```python
from build123d import *

# Parameters (mm, degrees)
SKETCH_1_W             = 42
SKETCH_1_H             = 54
EXTRUDE_1_DEPTH        = 55
SKETCH_5_W             = 65.5
SKETCH_5_H             = 65.5
EXTRUDE_3_DEPTH        = 8
SKETCH_6_R             = 10
EXTRUDE_4_DEPTH        = 5
HOLE_WIZARD_M4_1_D     = 3.3
HOLE_WIZARD_M4_1_DEPTH = 11.5
HOLE_WIZARD_M4_1_TIP   = 0.991420021
CHAMFER_1_SIZE         = 2
SKETCH_9_W             = 65.5
SKETCH_9_H             = 65.5
EXTRUDE_5_DEPTH        = 3
SKETCH_10_R            = 26
SKETCH_10_R_2          = 22.5
EXTRUDE_6_DEPTH        = 8
EXTRUDE_7_DEPTH        = 8
FILLET_1_R             = 2
FILLET_2_R             = 1
FILLET_3_R             = 0.8
SKETCH_12_R            = 1.5
CUT_EXTRUDE_1_DEPTH    = 1
CHAMFER_2_SIZE         = 2


with BuildPart() as part:
    # 草图1 → 凸台-拉伸1 (new body)
    with BuildSketch(Plane.XY):
        Rectangle(SKETCH_1_W, SKETCH_1_H)
    extrude(amount=EXTRUDE_1_DEPTH)

    # 草图5 → 凸台-拉伸3 (add)
    with BuildSketch(Plane.XY.offset(55)):
        Rectangle(SKETCH_5_W, SKETCH_5_H)
    extrude(amount=EXTRUDE_3_DEPTH)

    # 草图6 → 凸台-拉伸4 (add)
    with BuildSketch(Plane.XY.offset(63)):
        with Locations(Location((0, 0, 0), (0, 0, 180))):
            Circle(SKETCH_6_R)
    extrude(amount=EXTRUDE_4_DEPTH)

    # M4 螺纹孔1
    with Locations(Plane.XY.offset(63)):
        with Locations((-24, 24), (24, 24), (24, -24), (-24, -24)):
            Hole(HOLE_WIZARD_M4_1_D / 2, depth=HOLE_WIZARD_M4_1_DEPTH)
            with Locations((0, 0, -(HOLE_WIZARD_M4_1_DEPTH + HOLE_WIZARD_M4_1_TIP / 2))):  # 118° drill point
                Cone(0, HOLE_WIZARD_M4_1_D / 2, HOLE_WIZARD_M4_1_TIP, mode=Mode.SUBTRACT)

    # 倒角1
    chamfer_1_edges = [part.edges().sort_by_distance(p)[0] for p in [
        (32.75, -32.75, 59),
        (32.75, 32.75, 59),
        (-32.75, 32.75, 59),
        (-32.75, -32.75, 59),
    ]]
    chamfer(chamfer_1_edges, length=CHAMFER_1_SIZE)

    # 草图9 → 凸台-拉伸5 (add)
    with BuildSketch(Plane.XY.offset(68)):
        Rectangle(SKETCH_9_W, SKETCH_9_H)
    extrude(amount=EXTRUDE_5_DEPTH)

    # 草图10 → 凸台-拉伸6 (add)
    with BuildSketch(Plane.XY.offset(71)):
        with Locations(Location((0, 0, 0), (0, 0, 180))):
            Circle(SKETCH_10_R)
        Circle(SKETCH_10_R_2, mode=Mode.SUBTRACT)
    extrude(amount=EXTRUDE_6_DEPTH)

    # 草图11 → 凸台-拉伸7 (add)
    with BuildSketch(Plane.XY.offset(71)):
        with BuildLine():
            Line((2.781074433, 13.125), (6.952686082, 2.8125))
            ThreePointArc((6.952686082, 2.8125), (7.494884169, 0.276968033), (7.141306875, -2.291666667))
            Line((7.141306875, -2.291666667), (1.9043485, -18.611111111))
            ThreePointArc((1.9043485, -18.611111111), (0, -20), (-1.9043485, -18.611111111))
            Line((-1.9043485, -18.611111111), (-7.141306875, -2.291666667))
            ThreePointArc((-7.141306875, -2.291666667), (-7.494884169, 0.276968033), (-6.952686082, 2.8125))
            Line((-6.952686082, 2.8125), (-2.781074433, 13.125))
            ThreePointArc((-2.781074433, 13.125), (0, 15), (2.781074433, 13.125))
        make_face()
    extrude(amount=EXTRUDE_7_DEPTH)

    # 圆角1
    fillet_1_edges = [part.edges().sort_by_distance(p)[0] for p in [
        (26, 0, 71),
    ]]
    fillet(fillet_1_edges, radius=FILLET_1_R)

    # 圆角2
    fillet_2_edges = [part.edges().sort_by_distance(p)[0] for p in [
        (-22.5, 0, 71),
    ]]
    fillet(fillet_2_edges, radius=FILLET_2_R)

    # 圆角3
    fillet_3_edges = [part.edges().sort_by_distance(p)[0] for p in [
        (26, 0, 79),
        (-22.5, 0, 79),
    ]]
    fillet(fillet_3_edges, radius=FILLET_3_R)

    # 草图12 → 切除-拉伸1 (cut)
    with BuildSketch(Plane.XY.offset(79)):
        with Locations((0, 12)):
            Circle(SKETCH_12_R)
    extrude(amount=-CUT_EXTRUDE_1_DEPTH, mode=Mode.SUBTRACT)

    # 倒角2
    chamfer_2_edges = [part.edges().sort_by_distance(p)[0] for p in [
        (32.75, -32.75, 69.5),
        (32.75, 32.75, 69.5),
        (-32.75, 32.75, 69.5),
        (-32.75, -32.75, 69.5),
    ]]
    chamfer(chamfer_2_edges, length=CHAMFER_2_SIZE)


solid = part.part
```
Geometry: final body of the model. Coordinates: model frame, mm. A direction names the side the tool comes from. Give positions to 0.01 mm unless a question says otherwise; leave off trailing zeros. Order: outer loops, then holes, each group sorted by start corner. A loop starts at its lowest first (then second) coordinate and runs counter-clockwise, first axis right, second up. Notation, with made-up numbers: (-9.75, 25) -> (48.25, 25) arc R20 ccw to (48.25, 62) -> close; hole circle Ø6 at (89, 84). An arc over 180 degrees is marked (long way). Write each question's results on one line, items separated by ' | '. Start each with the question number.
1) Set-up query: faces 1 (the flat face through (-31.7, 31.8, 69.5)), 2 (the cylindrical face through (0, -20, 75)), 3 (the flat face through (21, 0, 27)), 4 (the flat face through (-21, 0, 27)), 5 (the cylindrical face through (-22.784, -22.885, 58.944)). Return all of +Z, -Z, +X, -X, +Y, -Y with unobstructed straight access to the full face (end or side cutting, diameter ignored); none if empty.
2) First-contact query: pin 1 (3 mm diameter, centred on x = -24, y = -24, fed in from -Z); pin 2 (4 mm diameter, centred on y = -12.5, z = 41, fed in from +X); pin 3 (6 mm diameter, centred on y = 21.5, z = 24, fed in from -X). Flat tips, straight axial feed; report the tip coordinate or a pass-through.
3) Draft query along X for faces 6 (the flat face through (31.8, 31.7, 58.9)), 7 (the flat face through (-7.3, 22.3, 79)), 8 (the cylindrical face through (10.382, -19.961, 75.057)). Return one class per face: pulls with the +X half, pulls with the -X half, needs draft (parallel to the pull), parting line crosses it, or undercut.
4) Line query: line 1 (Z direction, x = 1.5, y = -18.5); line 2 (Z direction, x = 19, y = 25); line 3 (Y direction, x = 0, z = 78.3). Output: solid intervals per line, ascending. Write a range as from..to.
5) Section A-A (z = 12.5). Return loops of the section in (x, y), then the cut area to 3 significant figures.
Calculated:
1) face 1: +Z, -Z, -X, +Y | face 2: +Z | face 3: -Z, +X, +Y, -Y | face 4: -Z, -X, +Y, -Y | face 5: -Z
2) pin 1: z = 68 | pin 2: x = 21 | pin 3: x = -21
3) face 6: pulls with the +X half | face 7: needs draft | face 8: undercut
4) line 1: 0..63, 68..79 | line 2: 0..63, 68..71 | line 3: -25.99..-22.51, -20..10.5, 13.5..15, 22.51..25.99
5) outline: (-21, -27) -> (21, -27) -> (21, 27) -> (-21, 27) -> close | area: 2,270 mm2
